Source: CAD feature listing. Evaluate the final solid. Frame: model axes, mm. A direction names the side the tool comes from. Give positions to 0.01 mm unless a question says otherwise; leave off trailing zeros. Write each loop counter-clockwise with the first axis right and the second up, starting at its lowest first coordinate (ties: lowest second). Pieces come first, ordered by that corner, then holes.
```python
from build123d import *

# Parameters (mm, degrees)
SKETCH1_R           = 50
SKETCH1_R_2         = 36
BOSS_EXTRUDE1_DEPTH = 15
CUT_EXTRUDE1_START  = -48
CUT_EXTRUDE1_DEPTH  = 48
SKETCH4_R           = 40
SKETCH4_R_2         = 30
BOSS_EXTRUDE2_DEPTH = 5
SKETCH5_R           = 43
SKETCH5_R_2         = 36
BOSS_EXTRUDE3_DEPTH = 33
SKETCH6_R           = 2
CUT_EXTRUDE2_DEPTH  = 30


with BuildPart() as part:
    # Sketch1 → Boss-Extrude1 (new body)
    with BuildSketch(Plane.XY):
        Circle(SKETCH1_R)
        Circle(SKETCH1_R_2, mode=Mode.SUBTRACT)
    extrude(amount=BOSS_EXTRUDE1_DEPTH)

    # Sketch2 → Cut-Extrude1 (cut)
    with BuildSketch(Plane.XY.offset(15).offset(CUT_EXTRUDE1_START)):
        with BuildLine():
            Line((-46.835, 17.506649451), (-46.835, -17.506649451))
            ThreePointArc((-46.835, -17.506649451), (-50, 0), (-46.835, 17.506649451))
        make_face()
        with BuildLine():
            Line((46.835, 17.506649451), (46.835, -17.506649451))
            ThreePointArc((46.835, -17.506649451), (50, 0), (46.835, 17.506649451))
        make_face()
    extrude(amount=CUT_EXTRUDE1_DEPTH, mode=Mode.SUBTRACT)

    # Sketch4 → Boss-Extrude2 (add)
    with BuildSketch(Plane(origin=(0, 0, 0), x_dir=(-1, 0, 0), z_dir=(0, 0, -1))):
        with Locations(Location((0, 0, 0), (0, 0, 180))):
            Circle(SKETCH4_R)
        Circle(SKETCH4_R_2, mode=Mode.SUBTRACT)
    extrude(amount=BOSS_EXTRUDE2_DEPTH)

    # Sketch5 → Boss-Extrude3 (add)
    with BuildSketch(Plane.XY.offset(15)):
        Circle(SKETCH5_R)
        Circle(SKETCH5_R_2, mode=Mode.SUBTRACT)
    extrude(amount=BOSS_EXTRUDE3_DEPTH)

    # Sketch6 → Cut-Extrude2 (cut)
    with BuildSketch(Plane.XY.offset(15)):
        with Locations((0, 46)):
            Circle(SKETCH6_R)
        with Locations((39.837168574, -23)):
            Circle(SKETCH6_R)
        with Locations((23, 39.837168574)):
            Circle(SKETCH6_R)
        with Locations((39.837168574, 23)):
            Circle(SKETCH6_R)
        with Locations((-23, 39.837168574)):
            Circle(SKETCH6_R)
        with Locations((-39.837168574, 23)):
            Circle(SKETCH6_R)
        with Locations((23, -39.837168574)):
            Circle(SKETCH6_R)
        with Locations((0, -46)):
            Circle(SKETCH6_R)
        with Locations((-23, -39.837168574)):
            Circle(SKETCH6_R)
        with Locations((-39.837168574, -23)):
            Circle(SKETCH6_R)
    extrude(amount=-CUT_EXTRUDE2_DEPTH, mode=Mode.SUBTRACT)


solid = part.part
```
1. Access query for faces 5 (the cylindrical face through (-23.26, -37.854, 7.605)), 6 (the flat face through (-14, -27, 0)). Directions: +Z, -Z, +X, -X, +Y, -Y. A direction counts if a zero-diameter tool reaches every point of the face in a straight line with its end or side. Return the directions, or none.
2. Cut plane A-A, the plane x = 0. Return the cut outline in (y, z).
3. Contact query for flat-ended pins moving along their axis: P1, Ø3.5, axis at x = -23, y = 39.84, coming from the -Z side; P2, Ø1.5, axis at x = 3.5, z = 39.5, coming from the +Y side; P3, Ø6.5, axis at x = -23, y = -39.84, coming from the -Z side; P4, Ø10, axis at x = -11, z = 12, coming from the -Y side. Output: stop coordinate, or through.
4. Cut plane B-B, the plane y = 0. Return the cut outline in (x, z) (3 decimals), then the cut area to 3 significant figures.
5. Cut plane D-D, the plane z = 11. State how many separate pieces and enclosed holes the cut face has, then the cut area to 3 significant figures.
6. Mould query, pull axis X, two halves, no side actions, for faces 1 (the cylindrical face through (-23.26, 41.82, 7.6)), 2 (the cylindrical face through (-0.849, -49.993, 7.395)), 3 (the flat face through (46.835, 0, 7)), 4 (the flat face through (-28, 30, 0)). Classes: +X half, -X half, draft (parallel to the pull), parting line (faces both ways), or undercut.
7. Cut plane C-C, the plane x = -9.5. Return the cut outline in (y, z).
8. Line query: L1, parallel to Y at x = 0, z = 12; L2, parallel to X at y = -22.5, z = 3; L3, parallel to Y at x = 0, z = -2. Output: solid intervals per line, ascending.
Response values:
1. face 5: +Z, -Z
1. face 6: +Z
2. outline: (-50, 0) - (-48, 0) - (-48, 15) - (-50, 15) - close; (-44, 0) - (-40, 0) - (-40, -5) - (-30, -5) - (-30, 0) - (-36, 0) - (-36, 48) - (-43, 48) - (-43, 15) - (-44, 15) - close; (30, -5) - (40, -5) - (40, 0) - (44, 0) - (44, 15) - (43, 15) - (43, 48) - (36, 48) - (36, 0) - (30, 0) - close; (48, 0) - (50, 0) - (50, 15) - (48, 15) - close
3. P1: passes through
3. P2: stops at y = 42.91
3. P3: stops at z = 0
3. P4: stops at y = -49.64
4. outline: (-46.835, 0) - (-40, 0) - (-40, -5) - (-30, -5) - (-30, 0) - (-36, 0) - (-36, 48) - (-43, 48) - (-43, 15) - (-46.835, 15) - close; (30, -5) - (40, -5) - (40, 0) - (46.835, 0) - (46.835, 15) - (43, 15) - (43, 48) - (36, 48) - (36, 0) - (30, 0) - close
4. area: 887 mm2
5. separate pieces: 1
5. enclosed holes: 11
5. area: 3,510 mm2
6. face 1: undercut
6. face 2: parting line
6. face 3: +X half
6. face 4: draft
7. outline: (-49.09, 0) - (-38.86, 0) - (-38.86, -5) - (-28.46, -5) - (-28.46, 0) - (-34.72, 0) - (-34.72, 48) - (-41.94, 48) - (-41.94, 15) - (-49.09, 15) - close; (28.46, -5) - (38.86, -5) - (38.86, 0) - (49.09, 0) - (49.09, 15) - (41.94, 15) - (41.94, 48) - (34.72, 48) - (34.72, 0) - (28.46, 0) - close
8. L1: y = -50 to -48, -44 to -36, 36 to 44, 48 to 50
8. L2: x = -44.65 to -41.77, -37.9 to -28.1, 28.1 to 37.9, 41.77 to 44.65
8. L3: y = -40 to -30, 30 to 40
